```python
from build123d import *

# Parameters (mm, degrees)
SKETCH2_W = 20
SKETCH2_H = 6


with BuildPart() as part:
    # Sweep1: sweep along a path in Sketch1
    with BuildLine(Plane.XY) as sweep1_path:
        Line((-460.524027919, 638.205508164), (92.975879138, 129.813393739))
        ThreePointArc((92.975879138, 129.813393739), (97.831928599, 99.10611839), (69.02602264, 87.412626283))
        Line((69.02602264, 87.412626283), (-652.122879897, 298.999368519))
        ThreePointArc((-652.122879897, 298.999368519), (-769.956329171, 589.271874597), (-460.524027919, 638.205508164))
    # Sketch2 → Sweep1 (sweep)
    with BuildSketch(Plane(origin=(-460.524027919, 0, 0), x_dir=(0, 0, -1), z_dir=(1, 0, 0))):
        with Locations((0, 635.205508164)):
            Rectangle(SKETCH2_W, SKETCH2_H)
    sweep(path=sweep1_path.line)


solid = part.part
```
Check sheet for the modelled part. Datum: model origin and axes. Units: mm. A direction names the side the tool comes from. Round coordinates to 2 decimals unless told otherwise and drop trailing zeros. Loops run counter-clockwise (first coordinate to the right, second up) from the corner with the lowest first, then second, coordinate; pieces in that order, holes last. Notation, with made-up numbers: (33, 87.25) - (41, 87.25) arc R21 ccw to (41, 106.25) - close; hole circle Ø10 at (48, 88.5). An arc over 180 degrees is marked (long way). Answer as a JSON object with one key per item and string values. Group by question number.
Q1. Gauge pin test, flat ends, axial feed: P1, Ø1.5, axis at y = 287.5, z = 7, coming from the +X side; P2, Ø5, axis at y = 519, z = 7.5, coming from the +X side; P3, Ø4, axis at x = -278.5, z = 3.5, coming from the +Y side. Record the tip position at first contact, or that the pin passes through.
Q2. Sectioned sample at C-C, the plane y = 198.5. Enter the section's corners in (x, z).
Q3. Sectioned sample at A-A, the plane x = -154.5. Enter the section's corners in (y, z), plus the area to 3 significant figures.
Q4. Sectioned sample at B-B, the plane z = 6.75. Enter the section's corners in (x, y), plus the area to 3 significant figures.
Q5. Set-up check for faces 1 (the face through (-412, 231, -10)), 2 (the face through (-299.25, 200.07, 0.14)): record each of +Z, -Z, +X, -X, +Y, -Y from which the full face is reachable in a straight line by a thin tool's end or side.
Q6. Mould release check, pull along Y, two halves, no side actions. Record for faces 3 (the face through (-345, 211, 10)), 4 (the face through (-766.57, 586.36, -0.14)), 5 (the face through (-179.9, 374.45, 0.14)), 6 (the face through (-296.6, 194.69, -0.14)): released by +Y, released by -Y, zero draft, split by the parting line, or undercut.
Q7. Scan lines: line 1 along Y through (x, z) = (-431, -6); line 2 along Y through (x, z) = (3, 0); line 3 along X through (y, z) = (666, -0.5). Record each from-to range of solid material in increasing order. Write a range as [from, to].
Solution:
{
 "1": {"P1": "stops at x = -77.89", "P2": "stops at x = -328.02", "P3": "stops at y = 472.85"},
 "2": {"outline": "(-309.59, -10) - (-293.9, -10) - (-293.9, 10) - (-309.59, 10) - close; (11.66, -10) - (18.19, -10) - (18.19, 10) - (11.66, 10) - close"},
 "3": {"outline": "(153, -10) - (157.6, -10) - (157.6, 10) - (153, 10) - close; (351.12, -10) - (357.12, -10) - (357.12, 10) - (351.12, 10) - close", "area": "212 mm²"},
 "4": {"outline": "(-652.12, 299) - (69.03, 87.41) arc R25 ccw to (92.98, 129.81) - (-460.52, 638.21) arc R200 ccw (long way) to start; hole (-654.77, 304.38) - (66.38, 92.8) arc R20.98 ccw to (92.98, 123.81) - (-460.52, 632.21) arc R195.62 ccw (long way) to start", "area": "10,000 mm²"},
 "5": {"face 1": "-Z, +X, -X, +Y, -Y", "face 2": "+Z, -Z"},
 "6": {"face 3": "zero draft", "face 4": "undercut", "face 5": "undercut", "face 6": "released by -Y"},
 "7": {"line 1": "y = [234.12, 238.73], [605.09, 611.09]", "line 2": "y = [106.78, 111.39], [206.46, 212.46]", "line 3": "x = [-692.48, -683.06], [-508.57, -499.15]"}
}
